Input: part model. Units: mm. Frame: model coordinates. A direction names the side the tool comes from. Give positions to 0.01 mm unless a question says otherwise; leave off trailing zeros. Loops run counter-clockwise (first coordinate to the right, second up) from the corner with the lowest first, then second, coordinate; pieces in that order, holes last. Notation, with made-up numbers: (8, -32.5) - (60, -32.5) arc R15 ccw to (60, -7.5) - close; hole circle Ø7 at (46.25, 83.25). An arc over 180 degrees is marked (long way). One line per item, written item: value.
from build123d import *

# Parameters (mm, degrees)
BOSS_EXTRUDE1_DEPTH     = 25
SKETCH2_R               = 2
CUT_EXTRUDE1_DEPTH      = 45.234732103
FILLET1_R               = 2
FILLET2_R               = 2
CUT_EXTRUDE2_START      = -6.5
SKETCH3_R               = 5
CUT_EXTRUDE2_DEPTH      = 6.5
SKETCH4_R               = 5
CUT_EXTRUDE3_DEPTH      = 6.5
CUT_EXTRUDE4_DEPTH      = 45.13919265
CUT_EXTRUDE4_DEPTH_BACK = 45.13919265
SKETCH5_W               = 10
SKETCH5_H               = 21
SKETCH5_W_2             = 12
SKETCH5_H_2             = 9
SKETCH7_W               = 8
SKETCH7_H               = 9
CUT_EXTRUDE5_DEPTH      = 2
CUT_EXTRUDE6_DEPTH      = 189.558524252
CUT_EXTRUDE6_DEPTH_BACK = 189.558524252
SKETCH8_R               = 1.5
CUT_EXTRUDE7_DEPTH      = 46.578505635
CUT_EXTRUDE7_DEPTH_BACK = 46.578505635
SKETCH9_W               = 12.618942776
SKETCH9_H               = 2


with BuildPart() as part:
    # Sketch1 → Boss-Extrude1 (new body)
    with BuildSketch(Plane(origin=(0, 0, 0), x_dir=(1, 0, 0), z_dir=(0, 1, 0))):
        with BuildLine():
            Line((-4.330127019, -2.5), (-10.330127019, -2.5))
            Line((-10.330127019, -2.5), (-4.911624974, -30.935916722))
            ThreePointArc((-4.911624974, -30.935916722), (0, -35), (4.911624974, -30.935916722))
            Line((4.911624974, -30.935916722), (10.330127019, -2.5))
            Line((10.330127019, -2.5), (4.330127019, -2.5))
            ThreePointArc((4.330127019, -2.5), (0, 5), (-4.330127019, -2.5))
        make_face()
    extrude(amount=BOSS_EXTRUDE1_DEPTH)

    # Sketch2 → Cut-Extrude1 (cut, through all)
    with BuildSketch(Plane(origin=(0, 25, 0), x_dir=(1, 0, 0), z_dir=(0, 1, 0))):
        with Locations(Location((0, 0, 0), (0, 0, 270))):
            Circle(SKETCH2_R)
        with Locations(Location((0, -30, 0), (0, 0, 270))):
            Circle(SKETCH2_R)
    extrude(amount=-CUT_EXTRUDE1_DEPTH, mode=Mode.SUBTRACT)

    # Fillet1
    fillet1_edges = [part.edges().sort_by_distance(p)[0] for p in [
        (10.330127019, 12.5, 2.5),
    ]]
    fillet(fillet1_edges, radius=FILLET1_R)

    # Fillet2
    fillet2_edges = [part.edges().sort_by_distance(p)[0] for p in [
        (-10.330127019, 12.5, 2.5),
    ]]
    fillet(fillet2_edges, radius=FILLET2_R)

    # Sketch3 → Cut-Extrude2 (cut)
    with BuildSketch(Plane(origin=(0, 25, 0), x_dir=(1, 0, 0), z_dir=(0, 1, 0)).offset(CUT_EXTRUDE2_START)):
        Circle(SKETCH3_R)
    extrude(amount=CUT_EXTRUDE2_DEPTH, mode=Mode.SUBTRACT)

    # Sketch4 → Cut-Extrude3 (cut)
    with BuildSketch(Plane.XZ):
        Circle(SKETCH4_R)
    extrude(amount=-CUT_EXTRUDE3_DEPTH, mode=Mode.SUBTRACT)

    # Sketch5 → Cut-Extrude4 (cut, two sides: drawn at the far end of the back side and taken through both)
    with BuildSketch(Plane(origin=(0, 0, 0), x_dir=(0, 0, -1), z_dir=(1, 0, 0)).offset(-CUT_EXTRUDE4_DEPTH_BACK)):
        with Locations((-30, 12.5)):
            Rectangle(SKETCH5_W, SKETCH5_H)
        with Locations((-1, 12.5)):
            Rectangle(SKETCH5_W_2, SKETCH5_H_2)
    extrude(amount=CUT_EXTRUDE4_DEPTH + CUT_EXTRUDE4_DEPTH_BACK, mode=Mode.SUBTRACT)

    # Sketch7 → Cut-Extrude5 (cut)
    with BuildSketch(Plane(origin=(10.427871309, 0, 1.987044855), x_dir=(0.18718334440142867, 0, -0.9823249948864665), z_dir=(0.9823249948864665, 0, 0.18718334440142867))):
        with Locations((-9.103153408, 12.5)):
            Rectangle(SKETCH7_W, SKETCH7_H)
    extrude(amount=-CUT_EXTRUDE5_DEPTH, mode=Mode.SUBTRACT)

    # Sketch8 → Cut-Extrude6 (cut, two sides: drawn at the far end of the back side and taken through both)
    with BuildSketch(Plane(origin=(59.598686513, 25, -138.486129663), x_dir=(0.989316462347077, 0, 0.14578387197857126), z_dir=(0, 1, 0)).offset(-CUT_EXTRUDE6_DEPTH_BACK)):
        with Locations(Location((-37.539914968, -158.208081577, 0), (0, 0, 278.382674106))):
            Circle(SKETCH8_R)
    extrude(amount=CUT_EXTRUDE6_DEPTH + CUT_EXTRUDE6_DEPTH_BACK, mode=Mode.SUBTRACT)

    # Sketch9 → Cut-Extrude7 (cut, two sides: drawn at the far end of the back side and taken through both)
    with BuildSketch(Plane(origin=(8.46322132, 0, 1.612678166), x_dir=(0.18718334440142864, 0, -0.9823249948864664), z_dir=(0.9823249948864664, 0, 0.18718334440142864)).offset(-CUT_EXTRUDE7_DEPTH_BACK)):
        with Locations((-11.793727477, 11.917152734)):
            Rectangle(SKETCH9_W, SKETCH9_H)
    extrude(amount=CUT_EXTRUDE7_DEPTH + CUT_EXTRUDE7_DEPTH_BACK, mode=Mode.SUBTRACT)


solid = part.part
Item 1: Draft query along Z for faces 4 (the face through (-0.37, 11.9, 18.36)), 5 (the face through (0, 12, 25)), 6 (the face through (6.714, 14.987, 10.795)), 7 (the face through (7.007, 9.438, 14.674)). Return one class per face: pulls with the +Z half, pulls with the -Z half, needs draft (parallel to the pull), parting line crosses it, or undercut.
Verdict:
face 4: pulls with the -Z half
face 5: pulls with the +Z half
face 6: undercut
face 7: undercut
Item 2: Material intervals for L1, parallel to Y at x = 4.5, z = 18.5; L2, parallel to Y at x = 1, z = -2.5; L3, parallel to Z at x = -1.75, y = 13.5, sorted ascending.
Verdict:
L1: y = 0 to 10.92, 12.92 to 25
L2: y = 6.5 to 8, 17 to 18.5
L3: z = 7 to 11.59, 13.53 to 25
Item 3: Section B-B, the plane y = 9.5. Output: boundary loops of the cut face in (x, z).
Verdict:
outline: (-9.47, 7) - (7.44, 7) - (6.01, 14.48) - (7.98, 14.86) - (6.04, 25) - (-6.04, 25) - close; hole circle Ø3 at (-0.6, 12.56)
Item 4: Section D-D, the plane x = -5.5. Output: boundary loops of the cut face in (y, z), and give its area (3 significant figures).
Verdict:
outline: (0, 2.5) - (8, 2.5) - (8, 7) - (10.92, 7) - (10.92, 17.38) - (12.92, 17.38) - (12.92, 7) - (17, 7) - (17, 2.5) - (25, 2.5) - (25, 27.85) - (23, 27.85) - (23, 25) - (2, 25) - (2, 27.85) - (0, 27.85) - close
area: 513 mm^2
Item 5: Section C-C, the plane x = -8.5. Output: boundary loops of the cut face in (y, z), and give its area (3 significant figures).
Verdict:
outline: (0, 2.59) - (8, 2.59) - (8, 7) - (10.92, 7) - (10.92, 12.1) - (0, 12.1) - close; (12.92, 7) - (17, 7) - (17, 2.59) - (25, 2.59) - (25, 12.1) - (12.92, 12.1) - close
area: 188 mm^2
Item 6: Section A-A, the plane z = 0. Output: boundary loops of the cut face in (x, y), and give its area (3 significant figures).
Verdict:
outline: (-5, 6.5) - (-2, 6.5) - (-2, 8) - (-5, 8) - close; (-5, 17) - (-2, 17) - (-2, 18.5) - (-5, 18.5) - close; (2, 6.5) - (5, 6.5) - (5, 8) - (2, 8) - close; (2, 17) - (5, 17) - (5, 18.5) - (2, 18.5) - close
area: 18.0 mm^2
Item 7: Pin query (flat end, axial travel): P1, Ø1, axis at x = -4, y = 15, coming from the +Z side; P2, Ø5, axis at x = 0, z = 0, coming from the +Y side; P3, Ø1, axis at x = 1, y = 17.5, coming from the -Z side. Return the tip coordinate at first contact, or that it passes through.
Verdict:
P1: stops at z = 25
P2: stops at y = 18.5
P3: stops at z = -4.97
Item 8: Access query for faces 1 (the face through (6.714, 9.479, 10.795)), 2 (the face through (-0.1, 23, 27.8)), 3 (the face through (-1, 9, 7)). Directions: +Z, -Z, +X, -X, +Y, -Y. A direction counts if a zero-diameter tool reaches every point of the face in a straight line with its end or side. Return the directions, or none.
Verdict:
face 1: +X
face 2: +Z, +X, -X
face 3: -Z, +X, -X
